Build history of the part. All positions in model axes, mm. A direction names the side the tool comes from. Coordinates: 2 decimals unless noted, no trailing zeros. Loops run counter-clockwise (first coordinate to the right, second up) from the corner with the lowest first, then second, coordinate; pieces in that order, holes last. Notation, with made-up numbers: M -7,30.25 L 50,30.25 A23 cw 50,68.25 Z; hole C 75,56 d6. An arc over 180 degrees is marked long. Write each question's results on one line, items separated by ' | '. Start each with the question number.
from build123d import *

# Parameters (mm, degrees)
SKETCH1_W           = 30
SKETCH1_H           = 30
BOSS_EXTRUDE1_DEPTH = 840
SKETCH2_W           = 24
SKETCH2_H           = 24
CUT_EXTRUDE1_DEPTH  = 840


with BuildPart() as part:
    # Sketch1 → Boss-Extrude1 (new body)
    with BuildSketch(Plane.XY):
        with Locations((3.8671875, 17.344389065)):
            Rectangle(SKETCH1_W, SKETCH1_H)
    extrude(amount=BOSS_EXTRUDE1_DEPTH)

    # Sketch2 → Cut-Extrude1 (cut)
    with BuildSketch(Plane.XY.offset(840)):
        with Locations((3.8671875, 17.344389065)):
            Rectangle(SKETCH2_W, SKETCH2_H)
    extrude(amount=-CUT_EXTRUDE1_DEPTH, mode=Mode.SUBTRACT)


solid = part.part
1. Wall check: line 1 along Y through (x, z) = (9, 633.5); line 2 along X through (y, z) = (17.25, 426). Give the ranges that are in metal, low to high.
2. Which spindle directions (+Z, -Z, +X, -X, +Y, -Y) get a long thin tool onto all of the face, cutting with end or side? Do faces 1 (the flat face through (-8.133, 17, 426)), 2 (the flat face through (4, 31, 840)). Say none if no direction does.
3. Band-saw the part on C-C, the plane y = 17.25. List the corners of the cut face in (x, z), plus the area to 3 significant figures.
4. Mould opens along Y. For faces 3 (the flat face through (4, 32.344, 414)), 4 (the flat face through (4, 29.344, 426)), 5 (the flat face through (-11.133, 17, 414)) say: +Y half, -Y half, draft (parallel to the pull), parting line (faces both ways), or undercut.
5. Pin check, flat tip, straight feed: pin 1 (6 mm diameter, centred on x = 5.5, y = 11, fed in from -Z) (3 decimals). Stop position of the tip, or through.
6. Band-saw the part on B-B, the plane x = -2.25. List the corners of the cut face in (y, z), plus the area to 3 significant figures.
7. Band-saw the part on A-A, the plane z = 96.5. List the corners of the cut face in (x, y), plus the area to 3 significant figures.
Checked values:
1) line 1: 2.34 to 5.34, 29.34 to 32.34 | line 2: -11.13 to -8.13, 15.87 to 18.87
2) face 1: +Z, -Z | face 2: +Z, +X, -X, +Y, -Y
3) outline: M -11.13,0 L -8.13,0 L -8.13,840 L -11.13,840 Z; M 15.87,0 L 18.87,0 L 18.87,840 L 15.87,840 Z | area: 5,040 mm²
4) face 3: +Y half | face 4: undercut | face 5: draft
5) pin 1: through
6) outline: M 2.34,0 L 5.34,0 L 5.34,840 L 2.34,840 Z; M 29.34,0 L 32.34,0 L 32.34,840 L 29.34,840 Z | area: 5,040 mm²
7) outline: M -11.13,2.34 L 18.87,2.34 L 18.87,32.34 L -11.13,32.34 Z; hole M -8.13,5.34 L 15.87,5.34 L 15.87,29.34 L -8.13,29.34 Z | area: 324 mm²
